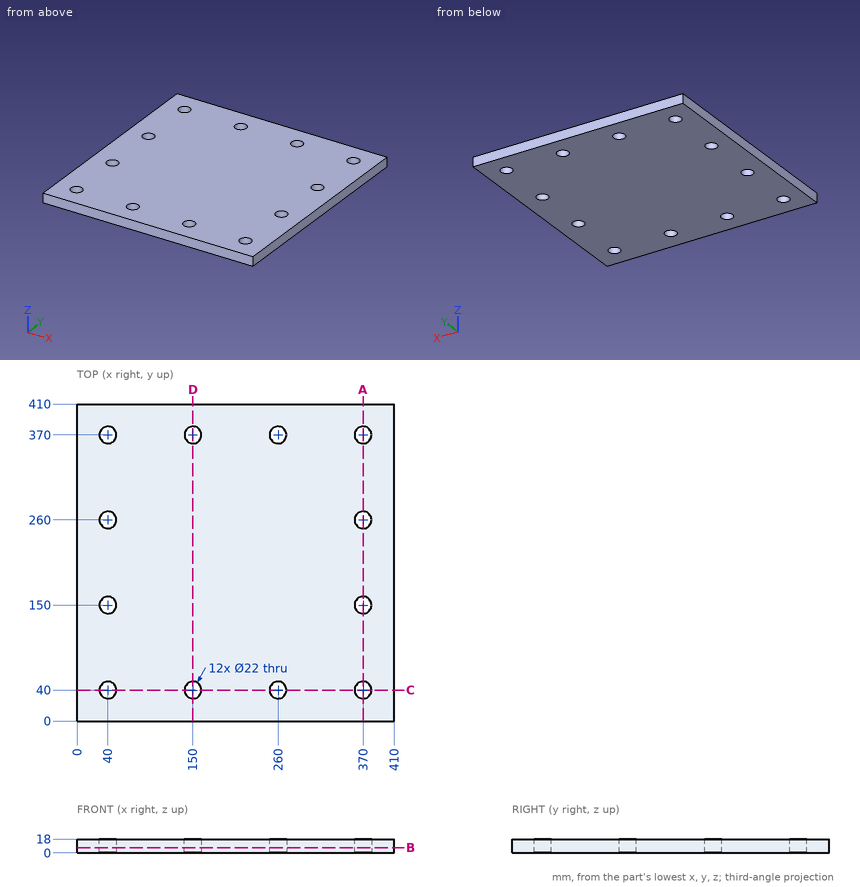
Job drawing, mm, ordinate dimensions from the low corner. One solid piece. Give positions to 0.01 mm unless a question says otherwise; leave off trailing zeros. Loops run counter-clockwise (first coordinate to the right, second up) from the corner with the lowest first, then second, coordinate; pieces in that order, holes last. Notation, with made-up numbers: M 55,45 L 91,45 A14 cw 91,53 Z; hole C -6,-32.75 d5. An arc over 180 degrees is marked long. Put each result on its own line as item: value. Start each with the question number.
1) Probe probe 1 along Y at (x, z) = (150, 4.5); probe 2 along Y at (x, z) = (39, 4). List the from-to ranges inside material, lowest first.
2) Saw through at D-D (x = 150). List the corners of the cut face in (y, z).
3) Saw through at A-A (x = 370). List the corners of the cut face in (y, z), then the cut area to 3 significant figures.
4) Saw through at B-B (z = 7). State how many separate pieces and enclosed holes the cut face has, then the cut area to 3 significant figures.
5) Flat gauge pins, fed straight in: pin 1 (20 mm diameter, centred on x = 260, y = 370, fed in from -Z); pin 2 (1 mm diameter, centred on x = 251.5, y = 128.5, fed in from -Z). Where does each tip first touch, or does it go through?
Numbers:
1. probe 1: 0 to 29, 51 to 359, 381 to 410
1. probe 2: 0 to 29.05, 50.95 to 139.05, 160.95 to 249.05, 270.95 to 359.05, 380.95 to 410
2. outline: M 0,0 L 29,0 L 29,18 L 0,18 Z; M 51,0 L 359,0 L 359,18 L 51,18 Z; M 381,0 L 410,0 L 410,18 L 381,18 Z
3. outline: M 0,0 L 29,0 L 29,18 L 0,18 Z; M 51,0 L 139,0 L 139,18 L 51,18 Z; M 161,0 L 249,0 L 249,18 L 161,18 Z; M 271,0 L 359,0 L 359,18 L 271,18 Z; M 381,0 L 410,0 L 410,18 L 381,18 Z
3. area: 5,800 mm^2
4. separate pieces: 1
4. enclosed holes: 12
4. area: 164,000 mm^2
5. pin 1: through
5. pin 2: z = 0
